Read the model definition and answer for the solid it produces. Units are mm, in the model's axes. Face numbers are marked on the shaded views. A direction names the side the tool comes from. Round coordinates to 2 decimals unless told otherwise and drop trailing zeros. Loops run counter-clockwise (first coordinate to the right, second up) from the corner with the lowest first, then second, coordinate; pieces in that order, holes last. Notation, with made-up numbers: (31.25, 13) -> (86.25, 13) arc R27 ccw to (86.25, 50) -> close; hole circle Ø7 at (-28, 67.5). An arc over 180 degrees is marked (long way). Put each result on its own line as item: value.
from build123d import *

# Parameters (mm, degrees)
CHAMFER1_SIZE = 0.5


with BuildPart() as part:
    # Sketch1 → Revolve1 (revolve)
    with BuildSketch(Plane.XY, mode=Mode.PRIVATE) as revolve1_sk:
        Polygon((380.5, -9.2), (380.5, -3.2), (385.5, -3.2), (385.5, -0.2), (380.5, -0.2), (380.5, 8), (375.5, 8), (375.5, 10.3), (368, 10.3), (368, -9.2), align=None)
    revolve(revolve1_sk.sketch.rotate(Axis((368, 10.3, 0), (0, -1, 0)), 90), axis=Axis((368, 10.3, 0), (0, -1, 0)))

    # Chamfer1
    chamfer1_edges = [part.edges().sort_by_distance(p)[0] for p in [
        (368, -0.2, -17.5),
        (368, -3.2, -17.5),
        (368, -9.2, -12.5),
        (368, 10.3, -7.5),
        (368, 8, -12.5),
    ]]
    chamfer(chamfer1_edges, length=CHAMFER1_SIZE)


solid = part.part
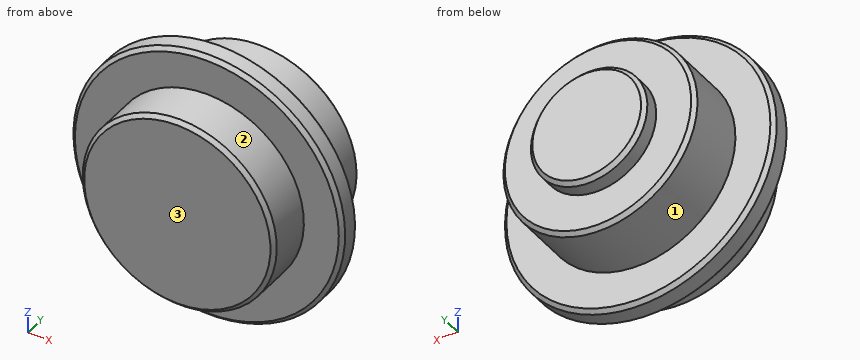
Item 1: Which of the six approach directions +Z, -Z, +X, -X, +Y, -Y give full straight-line access (tool end or side, diameter ignored) to the marked faces 1, 2 and 3?
Derived:
face 1: +Y
face 2: -Y
face 3: +Z, -Z, +X, -X, -Y
Item 2: The part is cut by section D-D (y = 8.75). Determine the outline of the cut face in (x, z).
Derived:
outline: circle Ø15 at (368, 0)
Item 3: The part is cut by section C-C (y = 2.75). Determine the outline of the cut face in (x, z), then the cut area to 3 significant figures.
Derived:
outline: circle Ø25 at (368, 0)
area: 491 mm^2
Item 4: The part is cut by section B-B (x = 368). Determine the outline of the cut face in (y, z), then the cut area to 3 significant figures.
Derived:
outline: (-9.2, -12) -> (-8.7, -12.5) -> (-3.2, -12.5) -> (-3.2, -17) -> (-2.7, -17.5) -> (-0.7, -17.5) -> (-0.2, -17) -> (-0.2, -12.5) -> (7.5, -12.5) -> (8, -12) -> (8, -7.5) -> (9.8, -7.5) -> (10.3, -7) -> (10.3, 7) -> (9.8, 7.5) -> (8, 7.5) -> (8, 12) -> (7.5, 12.5) -> (-0.2, 12.5) -> (-0.2, 17) -> (-0.7, 17.5) -> (-2.7, 17.5) -> (-3.2, 17) -> (-3.2, 12.5) -> (-8.7, 12.5) -> (-9.2, 12) -> close
area: 493 mm^2
Item 5: Find the intervals of material crossed by line 1 along Y through (x, z) = (376, 3); line 2 along Y through (x, z) = (364, -13); line 3 along Z through (x, y) = (368.5, -0.75), in increasing order.
Derived:
line 1: y = -9.2 to 8
line 2: y = -3.2 to -0.2
line 3: z = -17.49 to 17.49
Item 6: Flat-ended cylindrical pins translate along their axes: pin 1 Ø6 at (x, y) = (381, -1) entering from +Z; pin 2 Ø2 at (y, z) = (-2.5, -7) entering from +X; pin 3 Ø6 at (x, y) = (375, 7) entering from -Z. Find the tip coordinate at first contact, or state that the pin passes through.
Derived:
pin 1: stops at z = 14.36
pin 2: stops at x = 384.44
pin 3: stops at z = -11.84
Item 7: The part is cut by section A-A (z = 0). Determine the outline of the cut face in (x, y).
Derived:
outline: (350.5, -2.7) -> (351, -3.2) -> (355.5, -3.2) -> (355.5, -8.7) -> (356, -9.2) -> (380, -9.2) -> (380.5, -8.7) -> (380.5, -3.2) -> (385, -3.2) -> (385.5, -2.7) -> (385.5, -0.7) -> (385, -0.2) -> (380.5, -0.2) -> (380.5, 7.5) -> (380, 8) -> (375.5, 8) -> (375.5, 9.8) -> (375, 10.3) -> (361, 10.3) -> (360.5, 9.8) -> (360.5, 8) -> (356, 8) -> (355.5, 7.5) -> (355.5, -0.2) -> (351, -0.2) -> (350.5, -0.7) -> close
